Read the model definition and answer for the solid it produces. Units are mm, in the model's axes. A direction names the side the tool comes from. Give positions to 0.01 mm unless a question says otherwise; leave off trailing zeros. Write each loop counter-clockwise with the first axis right and the second up, starting at its lowest first coordinate (ties: lowest second). Pieces come first, ordered by that corner, then holes. Notation, with made-up numbers: M -11.5,-22 L 4.5,-22 A19 cw 4.5,-9 Z; hole C 13,17.25 d7. An arc over 180 degrees is marked long. Use a Markdown table: item, result. Add a question column.
Item 1: Given P1, Ø4, axis at x = 3.5, y = 0, coming from the +Z side; P2, Ø3, axis at x = 4, z = 7.5, coming from the +Y side; P3, Ø6, axis at y = 1.5, z = -12.5, coming from the +X side; P4, Ø1.5, axis at y = -5, z = -8.5, coming from the +X side, each flat-ended and moving along its own axis, determine where each tip first touches the part or whether it passes through.
Item 2: The mould has two halves that part along X. Classify faces 4 (the flat face through (0, 0, -18)), 5 (the flat face through (-2.465, 4.35, 10.463)), 6 (the cylindrical face through (-1.172, 8.923, 5.233)): pulls with the +X half, pulls with the -X half, needs draft (parallel to the pull), parting line crosses it, or undercut.
Item 3: A cutting plane is placed at A-A on z = 9.75. Determine the outline of the cut face in (x, y), then the cut area to 3 significant figures.
Item 4: A cutting plane is placed at C-C on z = -12.5. Determine the outline of the cut face in (x, y), then the cut area to 3 significant figures.
Item 5: A cutting plane is placed at B-B on z = 0.75. Determine the outline of the cut face in (x, y), then the cut area to 3 significant figures.
Item 6: Consider probe 1 along Z at (x, y) = (-6.25, -3); probe 2 along Y at (x, z) = (-1.75, 10.5); probe 3 along X at (y, z) = (5.25, 1). Determine where each line is inside the solid, lowest interval first. Write a range as [from, to].
Item 7: For faces 1 (the flat face through (-2, -5, 12)), 2 (the flat face through (2, -6, 0)), 3 (the flat face through (-2.535, -4.31, 10.463)), determine the directions among +Z, -Z, +X, -X, +Y, -Y from which every point of the face is accessible in a straight line to the end or side of a thin tool.
from build123d import *
from OCP.BRepFilletAPI import BRepFilletAPI_MakeChamfer

# Parameters (mm, degrees)
SKETCH1_R           = 9
BOSS_EXTRUDE1_DEPTH = 12
CUT_EXTRUDE1_DEPTH  = 6
SKETCH3_R           = 6
BOSS_EXTRUDE2_DEPTH = 18
CHAMFER1_SIZE       = 1.5
FILLET1_R           = 1.384615385
CHAMFER2_SIZE       = 2.88184438
CHAMFER2_SIZE2      = 4.991500886
FILLET2_R           = 0.1


with BuildPart() as part:
    # Sketch1 → Boss-Extrude1 (new body)
    with BuildSketch(Plane.XY):
        Circle(SKETCH1_R)
    extrude(amount=BOSS_EXTRUDE1_DEPTH)

    # Sketch2 → Cut-Extrude1 (cut)
    with BuildSketch(Plane.XY.offset(12)):
        Polygon((5, 2.886751346), (0, 5.773502692), (-5, 2.886751346), (-5, -2.886751346), (0, -5.773502692), (5, -2.886751346), align=None)
    extrude(amount=-CUT_EXTRUDE1_DEPTH, mode=Mode.SUBTRACT)

    # Sketch3 → Boss-Extrude2 (add)
    with BuildSketch(Plane(origin=(0, 0, 0), x_dir=(-1, 0, 0), z_dir=(0, 0, -1))):
        with Locations(Location((0, 0, 0), (0, 0, 180))):
            Circle(SKETCH3_R)
    extrude(amount=BOSS_EXTRUDE2_DEPTH)

    # Chamfer1
    chamfer1_edges = [part.edges().sort_by_distance(p)[0] for p in [
        (-6, 0, -18),
    ]]
    chamfer(chamfer1_edges, length=CHAMFER1_SIZE)

    # Fillet1
    fillet1_edges = [part.edges().sort_by_distance(p)[0] for p in [
        (-9, 0, 12),
    ]]
    fillet(fillet1_edges, radius=FILLET1_R)

    # Chamfer2: one chamfer whose edges measure the first distance from different faces: ONE call of the kernel's chamfer builder (chamfer() names one face for all edges)
    chamfer2_edges_1 = [part.edges().sort_by_distance(p)[0] for p in [
        (-2.5, 4.330127019, 6),
    ]]
    chamfer2_side_1 = [part.faces().sort_by_distance(p)[0] for p in [
        (-2.5, 4.330127019, 9),
    ]]
    chamfer2_edges_2 = [part.edges().sort_by_distance(p)[0] for p in [
        (2.5, 4.330127019, 6),
    ]]
    chamfer2_side_2 = [part.faces().sort_by_distance(p)[0] for p in [
        (2.5, 4.330127019, 9),
    ]]
    chamfer2_edges_3 = [part.edges().sort_by_distance(p)[0] for p in [
        (5, 0, 6),
    ]]
    chamfer2_side_3 = [part.faces().sort_by_distance(p)[0] for p in [
        (5, 0, 9),
    ]]
    chamfer2_edges_4 = [part.edges().sort_by_distance(p)[0] for p in [
        (2.5, -4.330127019, 6),
    ]]
    chamfer2_side_4 = [part.faces().sort_by_distance(p)[0] for p in [
        (2.5, -4.330127019, 9),
    ]]
    chamfer2_edges_5 = [part.edges().sort_by_distance(p)[0] for p in [
        (-2.5, -4.330127019, 6),
    ]]
    chamfer2_side_5 = [part.faces().sort_by_distance(p)[0] for p in [
        (-2.5, -4.330127019, 9),
    ]]
    chamfer2_edges_6 = [part.edges().sort_by_distance(p)[0] for p in [
        (-5, 0, 6),
    ]]
    chamfer2_side_6 = [part.faces().sort_by_distance(p)[0] for p in [
        (-5, 0, 9),
    ]]
    chamfer2 = BRepFilletAPI_MakeChamfer(part.part.solid().wrapped)
    for e in chamfer2_edges_1:
        chamfer2.Add(CHAMFER2_SIZE, CHAMFER2_SIZE2, e.wrapped, chamfer2_side_1[0].wrapped)  # the first distance lies on this face
    for e in chamfer2_edges_2:
        chamfer2.Add(CHAMFER2_SIZE, CHAMFER2_SIZE2, e.wrapped, chamfer2_side_2[0].wrapped)  # the first distance lies on this face
    for e in chamfer2_edges_3:
        chamfer2.Add(CHAMFER2_SIZE, CHAMFER2_SIZE2, e.wrapped, chamfer2_side_3[0].wrapped)  # the first distance lies on this face
    for e in chamfer2_edges_4:
        chamfer2.Add(CHAMFER2_SIZE, CHAMFER2_SIZE2, e.wrapped, chamfer2_side_4[0].wrapped)  # the first distance lies on this face
    for e in chamfer2_edges_5:
        chamfer2.Add(CHAMFER2_SIZE, CHAMFER2_SIZE2, e.wrapped, chamfer2_side_5[0].wrapped)  # the first distance lies on this face
    for e in chamfer2_edges_6:
        chamfer2.Add(CHAMFER2_SIZE, CHAMFER2_SIZE2, e.wrapped, chamfer2_side_6[0].wrapped)  # the first distance lies on this face
    add(Compound.cast(chamfer2.Shape()), mode=Mode.REPLACE)

    # Fillet2
    fillet2_edges = [part.edges().sort_by_distance(p)[0] for p in [
        (-6, 0, 0),
    ]]
    fillet(fillet2_edges, radius=FILLET2_R)


solid = part.part
Filled in:
| question | item | result |
|---|---|---|
| 1 | P1 | z = 12 |
| 1 | P2 | y = 8.65 |
| 1 | P3 | x = 6 |
| 1 | P4 | x = 4.24 |
| 2 | face 4 | needs draft |
| 2 | face 5 | undercut |
| 2 | face 6 | parting line crosses it |
| 3 | outline | C 0,0 d18; hole M -5,-2.89 L 0,-5.77 L 5,-2.89 L 5,2.89 L 0,5.77 L -5,2.89 Z |
| 3 | area | 168 mm² |
| 4 | outline | C 0,0 d12 |
| 4 | area | 113 mm² |
| 5 | outline | C 0,0 d18 |
| 5 | area | 254 mm² |
| 6 | probe 1 | [0, 12] |
| 6 | probe 2 | [-8.83, -4.76], [4.76, 8.83] |
| 6 | probe 3 | [-7.31, 7.31] |
| 7 | face 1 | +Z, +X, -X, +Y, -Y |
| 7 | face 2 | -Z |
| 7 | face 3 | +Z |
